Check sheet for the drawn part. Datum: minimum x, y, z corner. Units: mm. Round coordinates to 2 decimals unless told otherwise and drop trailing zeros. Order: outer loops, then holes, each group sorted by start corner. A loop starts at its lowest first (then second) coordinate and runs counter-clockwise, first axis right, second up. Notation, with made-up numbers: (82, 23.5) -> (113, 23.5) arc R30 ccw to (113, 57.5) -> close; hole circle Ø5 at (75.25, 14). An arc over 180 degrees is marked (long way). Use CSV: the item, a comma, the result in double quotes.
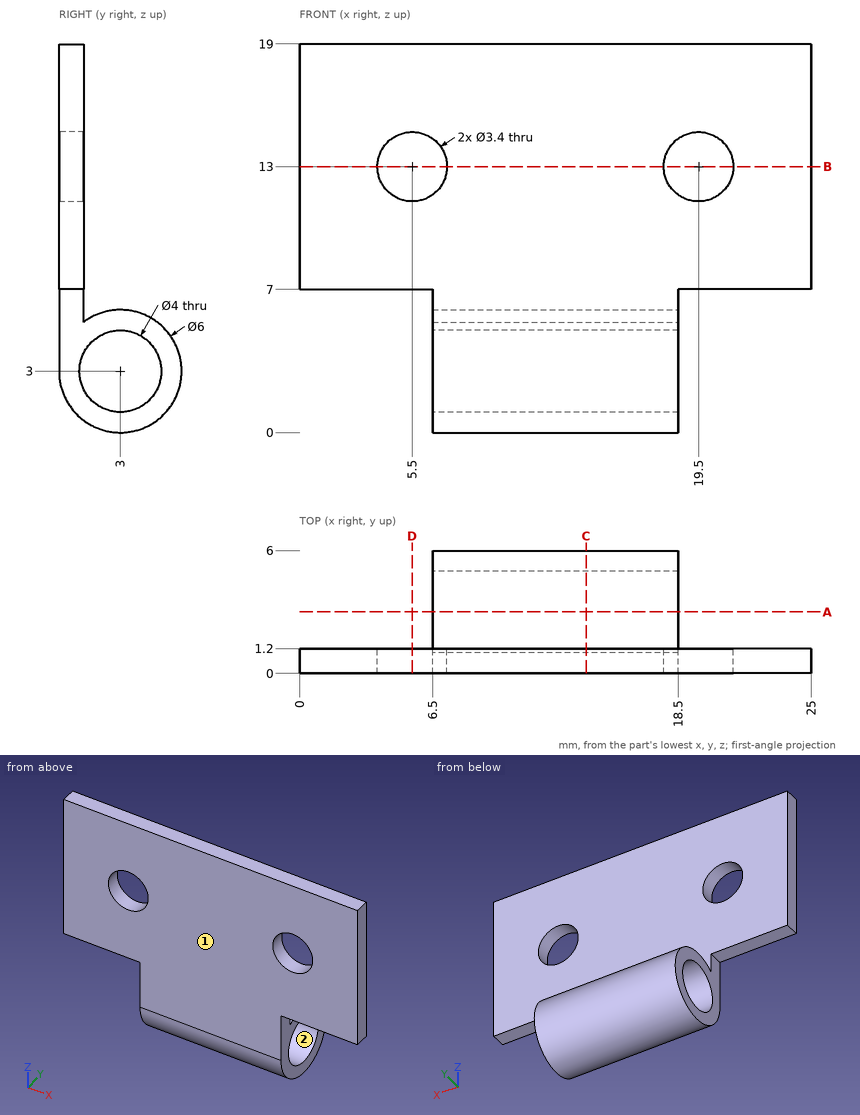
Q1. Sectioned sample at C-C, the plane x = 14. Enter the section's corners in (y, z).
Result sheet:
outline,"(0, 3) arc R3 ccw (long way) to (1.2, 5.4) -> (1.2, 19) -> (0, 19) -> close; hole circle Ø4 at (3, 3)"
Q2. Mould release check, pull along Y, two halves, no side actions. Record for the marked faces 1 and 2: pulls with the +Y half, pulls with the -Y half, needs draft (parallel to the pull), parting line crosses it, or undercut.
Result sheet:
face 1,"pulls with the -Y half"
face 2,"undercut"
Q3. Sectioned sample at A-A, the plane y = 3. Enter the section's corners in (x, z), then the cut area to 3 significant figures.
Result sheet:
outline,"(6.5, 0) -> (18.5, 0) -> (18.5, 1) -> (6.5, 1) -> close; (6.5, 5) -> (18.5, 5) -> (18.5, 6) -> (6.5, 6) -> close"
area,"24.0 mm^2"
Q4. Sectioned sample at B-B, the plane z = 13. Enter the section's corners in (x, y), then the cut area to 3 significant figures.
Result sheet:
outline,"(0, 0) -> (3.8, 0) -> (3.8, 1.2) -> (0, 1.2) -> close; (7.2, 0) -> (17.8, 0) -> (17.8, 1.2) -> (7.2, 1.2) -> close; (21.2, 0) -> (25, 0) -> (25, 1.2) -> (21.2, 1.2) -> close"
area,"21.8 mm^2"
Q5. Scan lines: L1, parallel to X at y = 0.8, z = 13; L2, parallel to Z at x = 16, y = 3; L3, parallel to Y at x = 13.25, z = 14.5. Record each from-to range of solid material in increasing order.
Result sheet:
L1,"x = 0 to 3.8, 7.2 to 17.8, 21.2 to 25"
L2,"z = 0 to 1, 5 to 6"
L3,"y = 0 to 1.2"
Q6. Sectioned sample at D-D, the plane x = 5.5. Enter the section's corners in (y, z).
Result sheet:
outline,"(0, 7) -> (1.2, 7) -> (1.2, 11.3) -> (0, 11.3) -> close; (0, 14.7) -> (1.2, 14.7) -> (1.2, 19) -> (0, 19) -> close"
Q7. Go/stop test with flat-tipped pins: pin 1 (0.6 mm diameter, centred on x = 22, y = 0.5, fed in from -Z); pin 2 (4.5 mm diameter, centred on x = 5.5, z = 13, fed in from +Y); pin 3 (1.5 mm diameter, centred on x = 17, z = 4, fed in from +Y); pin 4 (2 mm diameter, centred on x = 19.5, z = 13, fed in from +Y). Record where each tip stops, or that it passes through.
Result sheet:
pin 1,"stops at z = 7"
pin 2,"stops at y = 1.2"
pin 3,"stops at y = 5.99"
pin 4,"passes through"
